from build123d import *

# Parameters (mm, degrees)
EXTRUDE_1_DEPTH    = 8
HOLE_WIZARD_M3_1_D = 2.5
FILLET_1_R         = 0.5


with BuildPart() as part:
    # 草图1 → 凸台-拉伸1 (new body)
    with BuildSketch(Plane.XY):
        Polygon((-4, -16), (3, -16), (3, 0), (0, 0), (0, -13), (-4, -13), align=None)
    extrude(amount=EXTRUDE_1_DEPTH)

    # M3 螺纹孔1 (through all)
    with Locations(Plane(origin=(3, 0, 0), x_dir=(0, 0, -1), z_dir=(1, 0, 0))):
        with Locations((-4, -4)):
            Hole(HOLE_WIZARD_M3_1_D / 2)

    # 圆角1
    fillet_1_edges = [part.edges().sort_by_distance(p)[0] for p in [
        (-4, -13, 4),
        (-2, -13, 8),
        (-2, -13, 0),
    ]]
    fillet(fillet_1_edges, radius=FILLET_1_R)


solid = part.part
Read the model definition and answer for the solid it produces. Units are mm, in the model's axes. Coordinates: 2 decimals unless noted, no trailing zeros. Loops run counter-clockwise (first coordinate to the right, second up) from the corner with the lowest first, then second, coordinate; pieces in that order, holes last.
Q1. The part is cut by section D-D on z = 1.25. Write down the section's boundary in (x, y).
Q2. The part is cut by section C-C on x = 0.5. Write down the section's boundary in (y, z).
Q3. The part is cut by section A-A on z = 4. Write down the section's boundary in (x, y).
Q4. Consider probe 1 along Y at (x, z) = (2.1, 4); probe 2 along X at (y, z) = (-7.75, 4); probe 3 along Y at (x, z) = (-2, 6.5). Determine where each line is inside the solid, lowest interval first.
Q5. The mould has two halves that part along Y. Classify faces 1 (the face through (-2, -13, 4)), 2 (the face through (1.479, -5.109, 4.577)), 3 (the face through (1, -8, 8)): +Y half, -Y half, draft (parallel to the pull), parting line (faces both ways), or undercut.
Q6. This flat-tipped pin is pushed along its axis until it touches: pin 1 Ø3 at (x, y) = (-2.5, -8.5) entering from +Z. Where does it stop, or does it pass through?
Q7. The part is cut by section B-B on y = -4. Write down the section's boundary in (x, z), and give its area (3 significant figures).
Results below:
1. outline: (-4, -16) - (3, -16) - (3, 0) - (0, 0) - (0, -13) - (-3.5, -13) arc R0.5 ccw to (-4, -13.5) - close
2. outline: (-16, 0) - (0, 0) - (0, 8) - (-16, 8) - close; hole circle Ø2.5 at (-4, 4)
3. outline: (-4, -16) - (3, -16) - (3, -5.25) - (0, -5.25) - (0, -13) - (-3.5, -13) arc R0.5 ccw to (-4, -13.5) - close; (0, -2.75) - (3, -2.75) - (3, 0) - (0, 0) - close
4. probe 1: y = -16 to -5.25, -2.75 to 0
4. probe 2: x = 0 to 3
4. probe 3: y = -16 to -13
5. face 1: +Y half
5. face 2: undercut
5. face 3: draft
6. pin 1: passes through
7. outline: (0, 0) - (3, 0) - (3, 2.75) - (0, 2.75) - close; (0, 5.25) - (3, 5.25) - (3, 8) - (0, 8) - close
7. area: 16.5 mm2
